Part model, mm, in its own coordinate system. A direction names the side the tool comes from. Round coordinates to 2 decimals unless told otherwise and drop trailing zeros. Order: outer loops, then holes, each group sorted by start corner. A loop starts at its lowest first (then second) coordinate and runs counter-clockwise, first axis right, second up. Notation, with made-up numbers: (78.5, -21.5) - (93.5, -21.5) arc R19 cw to (93.5, 3.5) - close; hole circle Ø5 at (41, 75). An arc over 180 degrees is marked (long way). Answer as a JSON object with one key per item and string values.
```python
from build123d import *

# Parameters (mm, degrees)
BOSS_EXTRUDE1_DEPTH = 700


with BuildPart() as part:
    # Sketch1 → Boss-Extrude1 (new body)
    with BuildSketch(Plane.XY):
        with BuildLine():
            Line((0, 0), (295.706857871, 0))
            ThreePointArc((295.706857871, 0), (299.999011252, -0.046061756), (304.289187591, -0.184225806))
            Line((304.289187591, -0.184225806), (968.2, -28.7))
            Line((968.2, -28.7), (968.586204837, -19.708290161))
            Line((968.586204837, -19.708290161), (953.900403313, -12.071063335))
            Line((953.900403313, -12.071063335), (304.975773969, 15.801036129))
            ThreePointArc((304.975773969, 15.801036129), (300.342383522, 15.950253304), (295.706857871, 16))
            Line((295.706857871, 16), (30, 16))
            Line((30, 16), (0, 9))
            Line((0, 9), (0, 0))
        make_face()
    extrude(amount=BOSS_EXTRUDE1_DEPTH)


solid = part.part
```
Item 1: Drop flat-ended pins along their axis: P1, Ø1.5, axis at x = 710, z = 431, coming from the -Y side; P2, Ø12, axis at x = 574.5, z = 518.5, coming from the -Y side. Give the stop position or say it passes through.
Taken from the geometry:
{"P1": "y = -17.64", "P2": "y = -12.05"}
Item 2: Cut at C-C (x = 674.5). Write the cut outline in (y, z).
Taken from the geometry:
{"outline": "(-16.09, 0) - (-0.07, 0) - (-0.07, 700) - (-16.09, 700) - close"}
Item 3: Cut at A-A (z = 593.5). Write the cut outline in (x, y).
Taken from the geometry:
{"outline": "(0, 0) - (295.71, 0) arc R200 cw to (304.29, -0.18) - (968.2, -28.7) - (968.59, -19.71) - (953.9, -12.07) - (304.98, 15.8) arc R216 ccw to (295.71, 16) - (30, 16) - (0, 9) - close"}
Item 4: Tool access for faces 1 (the flat face through (15.21, 12.55, 345.1)), 2 (the flat face through (146, 0, 345)): list every direction of +Z, -Z, +X, -X, +Y, -Y with a clear straight run to the whole face (end or side of a thin tool).
Taken from the geometry:
{"face 1": "+Z, -Z, -X, +Y", "face 2": "+Z, -Z, -X, -Y"}
Item 5: Cut at B-B (x = 100.5). Write the cut outline in (y, z), plus the area to 3 significant figures.
Taken from the geometry:
{"outline": "(0, 0) - (16, 0) - (16, 700) - (0, 700) - close", "area": "11,200 mm2"}
Item 6: Probe L1, parallel to Y at x = 267, z = 445; L2, parallel to Y at x = 656.5, z = 152.5. List the from-to ranges inside material, lowest first. Write a range as from..to.
Taken from the geometry:
{"L1": "0..16", "L2": "-15.31..0.7"}
